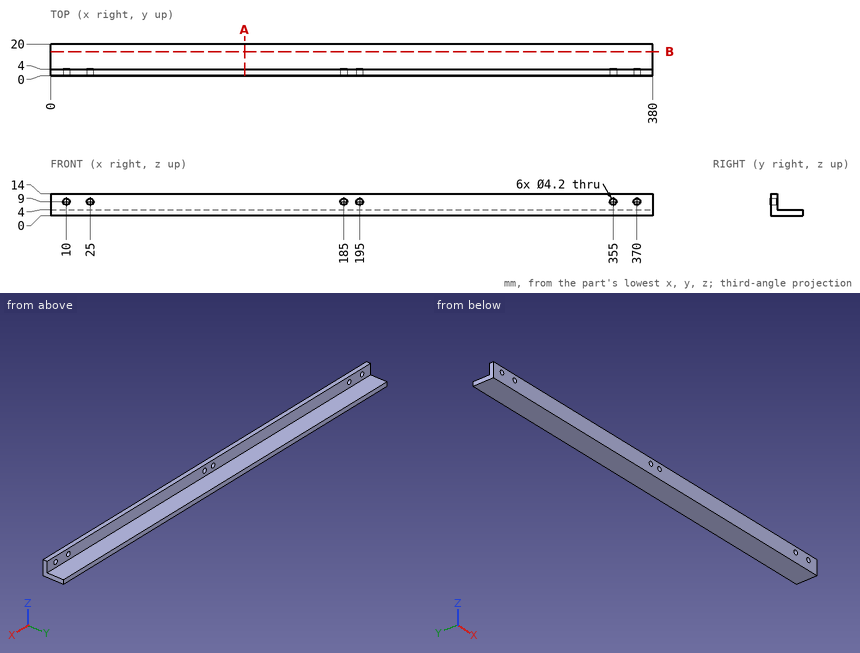
Here's the drawing with two shaded views (mm, measured from the low corner). I have some questions. Round coordinates to 2 decimals unless told otherwise and drop trailing zeros. Order: outer loops, then holes, each group sorted by start corner. A loop starts at its lowest first (then second) coordinate and runs counter-clockwise, first axis right, second up. Notation, with made-up numbers: M 18.5,57 L 55.5,57 A19 cw 55.5,76 Z; hole C -38,82 d7. An arc over 180 degrees is marked long. Answer in a Markdown table with one row per item.
Item 1: If I drill on L1, parallel to Z at x = 25, y = 2.1; L2, parallel to Z at x = 48.5, y = 6.5, over which ranges is the centre line in solid material (lowest first)? Write a range as from..to.
A:
| item | result |
|---|---|
| L1 | z = 0..6.9, 11.1..14 |
| L2 | z = 0..4 |
Item 2: Imagine slicing it at B-B, the plane y = 15.25. Write out the boundary of the cut face in (x, z), and give its area (3 significant figures).
A:
| item | result |
|---|---|
| outline | M 0,0 L 380,0 L 380,4 L 0,4 Z |
| area | 1,520 mm2 |
Item 3: Imagine slicing it at A-A, the plane x = 122.5. Write out the boundary of the cut face in (y, z), and give its area (3 significant figures).
A:
| item | result |
|---|---|
| outline | M 0,0 L 20,0 L 20,4 L 4,4 L 4,14 L 0,14 Z |
| area | 120 mm2 |
Item 4: I'm going to push flat-ended pins straight in: pin 1 (1 mm diameter, centred on x = 290.5, y = 7, fed in from +Z); pin 2 (5.5 mm diameter, centred on x = 370, z = 9, fed in from +Y). Where does each tip first touch, or does it pass through?
A:
| item | result |
|---|---|
| pin 1 | stops at z = 4 |
| pin 2 | stops at y = 4 |
